Work out the finished part from the listing and answer in its coordinate system (mm). Round coordinates to 2 decimals unless told otherwise and drop trailing zeros. Order: outer loops, then holes, each group sorted by start corner. A loop starts at its lowest first (then second) coordinate and runs counter-clockwise, first axis right, second up.
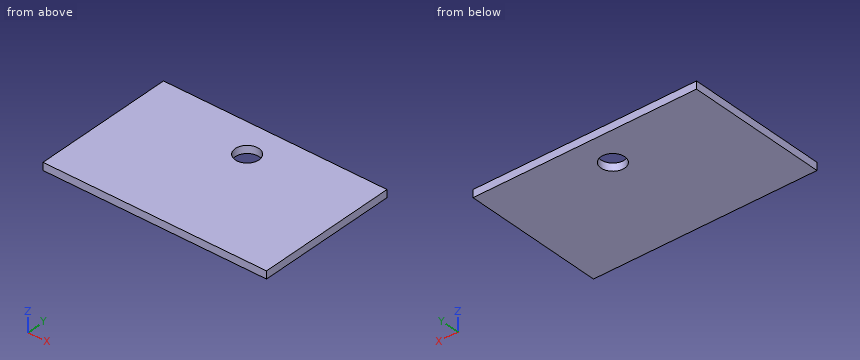
from build123d import *

# Parameters (mm, degrees)
SKETCH1_W                  = 236
SKETCH1_H                  = 150
BOSS_EXTRUDE1_DEPTH        = 4
F_25_0_25_DIAMETER_HOLE1_D = 25


with BuildPart() as part:
    # Sketch1 → Boss-Extrude1 (new, symmetric)
    with BuildSketch(Plane.XY):
        Rectangle(SKETCH1_W, SKETCH1_H)
    extrude(amount=BOSS_EXTRUDE1_DEPTH, both=True)

    # Ø25.0 (25) Diameter Hole1 (through all)
    with Locations(Plane.XY.offset(4)):
        with Locations((0, 40)):
            Hole(F_25_0_25_DIAMETER_HOLE1_D / 2)


solid = part.part
Item 1: Find section A-A (y = 40). Write down the section's boundary in (x, z).
Item 2: Find section B-B (x = 0). Write down the section's boundary in (y, z), plus the area to 3 significant figures.
Item 3: Find the intervals of material crossed by line 1 along X through (y, z) = (40.5, 0.5); line 2 along Y through (x, z) = (0, -1); line 3 along X through (y, z) = (49.5, 1), in increasing order.
Model answer:
1. outline: (-118, -4) - (-12.5, -4) - (-12.5, 4) - (-118, 4) - close; (12.5, -4) - (118, -4) - (118, 4) - (12.5, 4) - close
2. outline: (-75, -4) - (27.5, -4) - (27.5, 4) - (-75, 4) - close; (52.5, -4) - (75, -4) - (75, 4) - (52.5, 4) - close
2. area: 1,000 mm2
3. line 1: x = -118 to -12.49, 12.49 to 118
3. line 2: y = -75 to 27.5, 52.5 to 75
3. line 3: x = -118 to -8.12, 8.12 to 118
